Design review of the part built by this model. Coordinates are the model's own, in mm. A direction names the side the tool comes from. Round coordinates to 2 decimals unless told otherwise and drop trailing zeros. Write each loop counter-clockwise with the first axis right and the second up, starting at its lowest first coordinate (ties: lowest second). Pieces come first, ordered by that corner, then holes. Notation, with made-up numbers: M -13,-34.5 L 37,-34.5 A17 ccw 37,-13.5 Z; hole C 19,14 d4. An arc over 180 degrees is marked long. Use CSV: the item, a comma, the result in double quotes.
from build123d import *

# Parameters (mm, degrees)
SKETCH1_W           = 51
SKETCH1_H           = 8
BOSS_EXTRUDE1_DEPTH = 2
SKETCH2_R           = 1.75
CUT_EXTRUDE1_DEPTH  = 52.662365412
SKETCH3_R           = 4
BOSS_EXTRUDE2_DEPTH = 3
CHAMFER1_SIZE       = 0.5
CHAMFER2_SIZE       = 2


with BuildPart() as part:
    # Sketch1 → Boss-Extrude1 (new body)
    with BuildSketch(Plane(origin=(0, 0, 0), x_dir=(1, 0, 0), z_dir=(0, 1, 0))):
        with Locations((25.5, 4)):
            Rectangle(SKETCH1_W, SKETCH1_H)
    extrude(amount=BOSS_EXTRUDE1_DEPTH)

    # Sketch2 → Cut-Extrude1 (cut, through all)
    with BuildSketch(Plane(origin=(0, 2, 0), x_dir=(1, 0, 0), z_dir=(0, 1, 0))):
        with Locations(Location((5, 4, 0), (0, 0, 270))):
            Circle(SKETCH2_R)
    extrude(amount=-CUT_EXTRUDE1_DEPTH, mode=Mode.SUBTRACT)

    # Sketch3 → Boss-Extrude2 (add)
    with BuildSketch(Plane(origin=(0, 2, 0), x_dir=(1, 0, 0), z_dir=(0, 1, 0))):
        with Locations(Location((47, 4, 0), (0, 0, 270))):
            Circle(SKETCH3_R)
    extrude(amount=BOSS_EXTRUDE2_DEPTH)

    # Chamfer1
    chamfer1_edges = [part.edges().sort_by_distance(p)[0] for p in [
        (47, 5, -8),
    ]]
    chamfer(chamfer1_edges, length=CHAMFER1_SIZE)

    # Chamfer2
    chamfer2_edges = [part.edges().sort_by_distance(p)[0] for p in [
        (0, 1, -8),
        (51, 1, -8),
        (51, 1, 0),
        (0, 1, 0),
    ]]
    chamfer(chamfer2_edges, length=CHAMFER2_SIZE)


solid = part.part
1) Add section C-C on x = 33.5. Write out the cut boundary in (y, z).
Answers:
outline,"M 0,-8 L 2,-8 L 2,0 L 0,0 Z"
2) Add section A-A on y = 0.6. Write out the cut boundary in (x, z).
Answers:
outline,"M 0,-6 L 2,-8 L 49,-8 L 51,-6 L 51,-2 L 49,0 L 2,0 L 0,-2 Z; hole C 5,-4 d3.5"
3) Add section B-B on x = 5. Write out the cut boundary in (y, z), then the cut area to 3 significant figures.
Answers:
outline,"M 0,-8 L 2,-8 L 2,-5.75 L 0,-5.75 Z; M 0,-2.25 L 2,-2.25 L 2,0 L 0,0 Z"
area,"9.00 mm²"
4) For pin 1 Ø2.5 at (x, z) = (25.5, -6) entering from +Y; pin 2 Ø1.5 at (y, z) = (3.5, -6.5) entering from +X, all flat-tipped, find the tip position at first contact; note any pin that passes through.
Answers:
pin 1,"y = 2"
pin 2,"x = 50.6"
5) Machinability: for faces 4 (the face through (50, 1, -7)), 5 (the face through (43.451, 3.232, -2.154)), which of the approach directions +Z, -Z, +X, -X, +Y, -Y give a long, thin tool a straight path to every point of the face, cutting with its end or side? Answer none if there is none.
Answers:
face 4,"-Z, +X, +Y, -Y"
face 5,"+Y"
6) The part is to be moulded in two halves that separate along X. For faces 1 (the face through (3.94, 1.01, -5.39)), 2 (the face through (51, 1, -4)), 3 (the face through (25, 1, -8)), say which applies: released by +X, released by -X, zero draft, split by the parting line, or undercut.
Answers:
face 1,"undercut"
face 2,"released by +X"
face 3,"zero draft"
7) Add section D-D on y = 4. Write out the cut boundary in (x, z).
Answers:
outline,"C 47,-4 d8"
8) Wall thickness on line 1 along X through (y, z) = (1.2, -4); line 2 along Y through (x, z) = (10.5, -6.75); line 3 along Z through (x, y) = (4, 1.15): over which ranges is each line inside the solid? List them lowest first. Write a range as [from, to].
Answers:
line 1,"[0, 3.25], [6.75, 51]"
line 2,"[0, 2]"
line 3,"[-8, -5.44], [-2.56, 0]"
